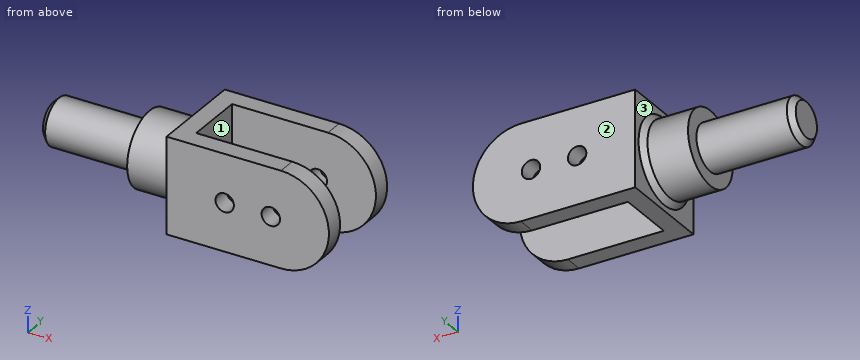
```python
from build123d import *

# Parameters (mm, degrees)
CLEVIS_BODY_52MM_DEPTH          = 52
ARM_END_BOSS_1_DEPTH            = 10
ARM_START                       = -10
ARM_END_BOSS_2_DEPTH            = 10
FORK_START                      = -70
FORK_TRIM_CUT_DEPTH             = 70
FORK_SLOT_PROFILE_W             = 26
FORK_SLOT_PROFILE_H             = 52
FORK_SLOT_CUT_DEPTH             = 70
ARM_END_BOSS_3_DEPTH            = 10
ARM_END_BOSS_4_DEPTH            = 10
COLLAR_PROFILE_R                = 20
COLLAR_25MM_DEPTH               = 25
COLLAR_CHAMFER_3X45_SIZE        = 3
SHANK_PROFILE_R                 = 12.5
SHANK_52MM_DEPTH                = 52
SHANK_END_CHAMFER_3X45_SIZE     = 3
PIN_HOLES_PROFILE_R             = 5
PIN_HOLES_2X_THROUGH_ARMS_DEPTH = 52


with BuildPart() as part:
    # Clevis Body Profile → Clevis Body 52mm (new body)
    with BuildSketch(Plane.XY):
        Polygon((0, 0), (88, 0), (88, -10), (10, -10), (10, -42), (88, -42), (88, -52), (0, -52), align=None)
    extrude(amount=CLEVIS_BODY_52MM_DEPTH)

    # Arm End Boss 1 Profile → Arm End Boss 1 (add)
    with BuildSketch(Plane(origin=(0, 0, 0), x_dir=(1, 0, 0), z_dir=(0, 1, 0))):
        with BuildLine():
            Line((88, 0), (88, -52))
            ThreePointArc((88, -52), (114, -26), (88, 0))
        make_face()
    extrude(amount=-ARM_END_BOSS_1_DEPTH)

    # Arm End Boss 2 Profile → Arm End Boss 2 (add)
    with BuildSketch(Plane.XZ.offset(52).offset(ARM_START)):
        with BuildLine():
            Line((88, 52), (88, 0))
            ThreePointArc((88, 0), (114, 26), (88, 52))
        make_face()
    extrude(amount=ARM_END_BOSS_2_DEPTH)

    # Fork Trim Cut Profile → Fork Trim Cut (cut)
    with BuildSketch(Plane.XZ.offset(52).offset(FORK_START)):
        with BuildLine():
            Line((88, 52), (88, 0))
            ThreePointArc((88, 0), (114, 26), (88, 52))
        make_face()
    extrude(amount=FORK_TRIM_CUT_DEPTH, mode=Mode.SUBTRACT)

    # Fork Slot Profile → Fork Slot Cut (cut)
    with BuildSketch(Plane.XZ.offset(52)):
        with Locations((75, 26)):
            Rectangle(FORK_SLOT_PROFILE_W, FORK_SLOT_PROFILE_H)
    extrude(amount=-FORK_SLOT_CUT_DEPTH, mode=Mode.SUBTRACT)

    # Arm End Boss 3 Profile → Arm End Boss 3 (add)
    with BuildSketch(Plane.XZ.offset(52)):
        with BuildLine():
            Line((62, 52), (62, 0))
            ThreePointArc((62, 0), (88, 26), (62, 52))
        make_face()
    extrude(amount=-ARM_END_BOSS_3_DEPTH)

    # Arm End Boss 4 Profile → Arm End Boss 4 (add)
    with BuildSketch(Plane(origin=(0, 0, 0), x_dir=(1, 0, 0), z_dir=(0, 1, 0)).offset(ARM_START)):
        with BuildLine():
            Line((62, 0), (62, -52))
            ThreePointArc((62, -52), (88, -26), (62, 0))
        make_face()
    extrude(amount=ARM_END_BOSS_4_DEPTH)

    # Collar Profile → Collar 25mm (add)
    with BuildSketch(Plane.ZY):
        with Locations((26, -26)):
            Circle(COLLAR_PROFILE_R)
    extrude(amount=COLLAR_25MM_DEPTH)

    # Collar Chamfer 3x45
    collar_chamfer_3x45_edges = [part.edges().sort_by_distance(p)[0] for p in [
        (0, -26, 6),
    ]]
    chamfer(collar_chamfer_3x45_edges, length=COLLAR_CHAMFER_3X45_SIZE)

    # Shank Profile → Shank 52mm (add)
    with BuildSketch(Plane.ZY.offset(25)):
        with Locations(Location((26, -26, 0), (0, 0, 180))):
            Circle(SHANK_PROFILE_R)
    extrude(amount=SHANK_52MM_DEPTH)

    # Shank End Chamfer 3x45
    shank_end_chamfer_3x45_edges = [part.edges().sort_by_distance(p)[0] for p in [
        (-77, -26, 38.5),
    ]]
    chamfer(shank_end_chamfer_3x45_edges, length=SHANK_END_CHAMFER_3X45_SIZE)

    # Pin Holes Profile → Pin Holes 2x Through Arms (cut)
    with BuildSketch(Plane.XZ.offset(52)):
        with Locations(Location((31.5, 26, 0), (0, 0, 270))):
            Circle(PIN_HOLES_PROFILE_R)
        with Locations(Location((56.5, 26, 0), (0, 0, 270))):
            Circle(PIN_HOLES_PROFILE_R)
    extrude(amount=-PIN_HOLES_2X_THROUGH_ARMS_DEPTH, mode=Mode.SUBTRACT)


solid = part.part
```
Geometry: final body of the model. Coordinates: model frame, mm. Face numbers are marked on the shaded views. A direction names the side the tool comes from. Give positions to 0.01 mm unless a question says otherwise; leave off trailing zeros. Write each loop counter-clockwise with the first axis right and the second up, starting at its lowest first coordinate (ties: lowest second). Pieces come first, ordered by that corner, then holes.
1. Line query: probe 1 along X at (y, z) = (-9, 26); probe 2 along X at (y, z) = (-2, 26); probe 3 along Y at (x, z) = (72, 43). Output: solid intervals per line, ascending.
2. Pin query (flat end, axial travel): P1, Ø10, axis at y = -46.5, z = 31.5, coming from the +X side; P2, Ø2, axis at y = -18.5, z = 8.5, coming from the +X side; P3, Ø8, axis at x = 31.5, z = 26, coming from the -Y side; P4, Ø1.5, axis at y = -11.5, z = 14, coming from the -X side. Return the tip coordinate at first contact, or that it passes through.
3. Section query A-A, the plane x = 56.5. Return loops of the section in (y, z).
4. Section query C-C, the plane x = 77. Return loops of the section in (y, z), then the cut area to 3 significant figures.
5. Reachability of the marked faces 1, 2 and 3 from +Z, -Z, +X, -X, +Y, -Y: full face, straight path, thin tool, end or side. Return the list, or none.
6. Section query B-B, the plane y = -26. Return loops of the section in (x, z).
7. Section query D-D, the plane z = 26. Count the separate pieces of the cut face and the enclosed holes in it, then the cut area to 3 significant figures.
Computed:
1. probe 1: x = -25 to 26.5, 36.5 to 51.5, 61.5 to 88
1. probe 2: x = 0 to 26.5, 36.5 to 51.5, 61.5 to 88
1. probe 3: y = -52 to -42, -10 to 0
2. P1: stops at x = 88
2. P2: stops at x = 10
2. P3: passes through
2. P4: stops at x = -25
3. outline: (-52, 0) - (-42, 0) - (-42, 21) - (-52, 21) - close; (-52, 31) - (-42, 31) - (-42, 52) - (-52, 52) - close; (-10, 0) - (0, 0) - (0, 21) - (-10, 21) - close; (-10, 31) - (0, 31) - (0, 52) - (-10, 52) - close
4. outline: (-52, 4.76) - (-42, 4.76) - (-42, 47.24) - (-52, 47.24) - close; (-10, 4.76) - (0, 4.76) - (0, 47.24) - (-10, 47.24) - close
4. area: 849 mm2
5. face 1: +Z, -Z, +X
5. face 2: +Z, -Z, +X, -X, +Y
5. face 3: -X
6. outline: (-77, 16.5) - (-74, 13.5) - (-25, 13.5) - (-25, 6) - (-3, 6) - (0, 3) - (0, 0) - (10, 0) - (10, 52) - (0, 52) - (0, 49) - (-3, 46) - (-25, 46) - (-25, 38.5) - (-74, 38.5) - (-77, 35.5) - close
7. separate pieces: 5
7. enclosed holes: 0
7. area: 3,980 mm2
